from build123d import *

# Parameters (mm, degrees)
SKETCH_1_R          = 1.7
EXTRUDE_1_DEPTH     = 5.998531593
SKETCH_2_R          = 1.5
EXTRUDE_2_DEPTH     = 10
SKETCH_3_R          = 2.5
EXTRUDE_3_DEPTH     = 4
CUT_EXTRUDE_1_DEPTH = 3


with BuildPart() as part:
    # 草图1 → 凸台-拉伸1 (new body)
    with BuildSketch(Plane.XY):
        with Locations((0, -6)):
            Circle(SKETCH_1_R)
    extrude(amount=-EXTRUDE_1_DEPTH)

    # 草图2 → 凸台-拉伸2 (add)
    with BuildSketch(Plane(origin=(0, 0, -5.998531593), x_dir=(-1, 0, 0), z_dir=(0, 0, -1))):
        with Locations(Location((0, -6, 0), (0, 0, 90))):
            Circle(SKETCH_2_R)
    extrude(amount=EXTRUDE_2_DEPTH)

    # 草图3 → 凸台-拉伸3 (add)
    with BuildSketch(Plane.XY):
        with Locations((0, -6)):
            Circle(SKETCH_3_R)
    extrude(amount=EXTRUDE_3_DEPTH)

    # 草图4 → 切除-拉伸1 (cut)
    with BuildSketch(Plane.XY.offset(4)):
        Polygon((1.355554736, -4.921820351), (-0.255953598, -4.286965337), (-1.611508335, -5.365144986), (-1.355554737, -7.078179649), (0.255953597, -7.713034663), (1.611508334, -6.634855014), align=None)
    extrude(amount=-CUT_EXTRUDE_1_DEPTH, mode=Mode.SUBTRACT)


solid = part.part
Geometry: final body of the model. Coordinates: model frame, mm. A direction names the side the tool comes from. Coordinates: 2 decimals unless noted, no trailing zeros. Order: outer loops, then holes, each group sorted by start corner. A loop starts at its lowest first (then second) coordinate and runs counter-clockwise, first axis right, second up.
(1) First-contact query: pin 1 (1.5 mm diameter, centred on y = -5, z = -0.5, fed in from -X); pin 2 (2 mm diameter, centred on y = -4, z = -11, fed in from -X); pin 3 (1 mm diameter, centred on x = -0.5, y = -4, fed in from -Z). Flat tips, straight axial feed; report the tip coordinate or a pass-through.
(2) Draft query along X for faces 1 (the face through (-0.33, -3.52, 1.97)), 2 (the face through (-0.56, -7.39, 2.52)), 3 (the face through (2, -7, 0)). Return one class per face: pulls with the +X half, pulls with the -X half, needs draft (parallel to the pull), parting line crosses it, or undercut.
(3) Section query D-D (x = 0). Return the cut outline in (y, z), plus the area to 3 significant figures.
(4) Section query A-A (z = 2). Return the cut outline in (x, y).
(5) Access query for faces 4 (the face through (0.07, -7.5, -10.93)), 5 (the face through (1.485, -5.79, 2.521)), 6 (the face through (0, -6, -15.999)). Directions: +Z, -Z, +X, -X, +Y, -Y. A direction counts if a zero-diameter tool reaches every point of the face in a straight line with its end or side. Return the directions, or none.
(6) Section query B-B (y = -6.9). Return the cut outline in (x, z).
(7) Material intervals for probe 1 along Z at (x, y) = (1.3, -5.5); probe 2 along Z at (x, y) = (2.1, -5.2); probe 3 along X at (y, z) = (-5.35, 2), sorted ascending.
(8) Section query C-C (z = -13.75). Return the cut outline in (x, y).
Solution:
1. pin 1: stops at x = -2.46
1. pin 2: stops at x = -1.12
1. pin 3: stops at z = -6
2. face 1: parting line crosses it
2. face 2: undercut
2. face 3: needs draft
3. outline: (-8.5, 0) - (-7.7, 0) - (-7.7, -6) - (-7.5, -6) - (-7.5, -16) - (-4.5, -16) - (-4.5, -6) - (-4.3, -6) - (-4.3, 0) - (-3.5, 0) - (-3.5, 4) - (-4.39, 4) - (-4.39, 1) - (-7.61, 1) - (-7.61, 4) - (-8.5, 4) - close
3. area: 60.7 mm2
4. outline: circle Ø5 at (0, -6); hole (-1.61, -5.37) - (-1.36, -7.08) - (0.26, -7.71) - (1.61, -6.63) - (1.36, -4.92) - (-0.26, -4.29) - close
5. face 4: -Z
5. face 5: +Z
5. face 6: -Z, +X, -X, +Y, -Y
6. outline: (-2.33, 0) - (-1.44, 0) - (-1.44, -6) - (-1.2, -6) - (-1.2, -16) - (1.2, -16) - (1.2, -6) - (1.44, -6) - (1.44, 0) - (2.33, 0) - (2.33, 4) - (1.28, 4) - (1.28, 1) - (-1.38, 1) - (-1.38, 4) - (-2.33, 4) - close
7. probe 1: z = -16 to 1
7. probe 2: z = 0 to 4
7. probe 3: x = -2.41 to -1.59, 1.42 to 2.41
8. outline: circle Ø3 at (0, -6)
